from build123d import *

# Parameters (mm, degrees)
BASE_PLATE_DEPTH            = 7
ANGLED_BLOCK_DEPTH          = 50
BLOCK_NOTCH_CUT_DEPTH       = 74.464277033
BLOCK_NOTCH_CUT_DEPTH_BACK  = 74.464277033
BLOCK_RECESS_CUT_DEPTH      = 72.480306495
BLOCK_RECESS_CUT_DEPTH_BACK = 13
BLOCK_RECESS_SKETCH_R       = 4


with BuildPart() as part:
    # Base Plate Sketch → Base Plate (new body)
    with BuildSketch(Plane.XY):
        Polygon((-44, 25), (-38, 31), (38, 31), (44, 25), (44, -25), (38, -31), (-38, -31), (-44, -25), align=None)
        with BuildLine():
            Line((-30, 20.5), (-30, -20.5))
            ThreePointArc((-30, -20.5), (-33, -23.5), (-36, -20.5))
            Line((-36, -20.5), (-36, 20.5))
            ThreePointArc((-36, 20.5), (-33, 23.5), (-30, 20.5))
        make_face(mode=Mode.SUBTRACT)
        with BuildLine():
            Line((36, 20.5), (36, -20.5))
            ThreePointArc((36, -20.5), (33, -23.5), (30, -20.5))
            Line((30, -20.5), (30, 20.5))
            ThreePointArc((30, 20.5), (33, 23.5), (36, 20.5))
        make_face(mode=Mode.SUBTRACT)
    extrude(amount=BASE_PLATE_DEPTH)

    # Angled Block Sketch → Angled Block (add)
    with BuildSketch(Plane.XY):
        Polygon((-19.704957389, -4.000247215), (-12.317392569, -15.892424729), (23.166882613, 6.150837127), (15.779317794, 18.043014641), align=None)
    extrude(amount=ANGLED_BLOCK_DEPTH)

    # Block Notch Sketch → Block Notch Cut (cut, two sides: drawn at the far end of the back side and taken through both)
    with BuildSketch(Plane(origin=(0, 0, 0), x_dir=(0.8494412510349073, 0.5276832014004726, 0), z_dir=(0.5276832014004726, -0.8494412510349073, 0)).offset(-BLOCK_NOTCH_CUT_DEPTH_BACK)):
        Polygon((-18.849066913, 50), (-18.849066913, 7), (22.924599176, 42.643551505), (22.924599176, 50), align=None)
        Polygon((10.753136621, 27), (10.753136621, 7), (15.483777963, 7), (22.924599176, 7), (22.924599176, 37.385350224), align=None)
    extrude(amount=BLOCK_NOTCH_CUT_DEPTH + BLOCK_NOTCH_CUT_DEPTH_BACK, mode=Mode.SUBTRACT)

    # Block Recess Sketch → Block Recess Cut (cut, two sides: drawn at the far end of the back side and taken through both)
    with BuildSketch(Plane(origin=(-9.681672009, -6.014372005, 13.357913864), x_dir=(0.8342680576474281, -0.22636189915410374, 0.5027495386378142), z_dir=(-0.5513590554159673, -0.3425109283644645, 0.7607164096834806)).offset(-BLOCK_RECESS_CUT_DEPTH_BACK)):
        with Locations(Location((29.524664999, 24.110272289, 0), (0, 0, 193.941739612))):
            Circle(BLOCK_RECESS_SKETCH_R)
        with BuildLine():
            ThreePointArc((36.524664999, 24.110272289), (35.848943941, 21.109689701), (33.952237609, 18.688409068))
            Line((33.952237609, 18.688409068), (39.374100831, 23.115981696))
            Line((39.374100831, 23.115981696), (34.946528251, 28.53784486))
            ThreePointArc((34.946528251, 28.53784486), (36.118337828, 26.460480496), (36.524664999, 24.110272289))
        make_face()
        with BuildLine():
            Line((30.518955591, 33.959708121), (25.097092428, 29.532135541))
            ThreePointArc((25.097092428, 29.532135541), (30.227734682, 31.07487515), (34.946528251, 28.53784486))
            Line((34.946528251, 28.53784486), (30.518955591, 33.959708121))
        make_face()
    extrude(amount=BLOCK_RECESS_CUT_DEPTH + BLOCK_RECESS_CUT_DEPTH_BACK, mode=Mode.SUBTRACT)


solid = part.part
Geometry check sheet. Reference: the model listing, model coordinates, mm. A direction names the side the tool comes from. Coordinates: 2 decimals unless noted, no trailing zeros. Loops run counter-clockwise (first coordinate to the right, second up) from the corner with the lowest first, then second, coordinate; pieces in that order, holes last. Notation, with made-up numbers: (8, 40) - (49, 40) arc R19 ccw to (49, 59) - close; hole circle Ø3 at (-34.75, 22). An arc over 180 degrees is marked (long way). Use one line per item in the form item = value. Start each with the question number.
Item 1: Section check D-D, the plane y = -13. Enter the section's corners in (x, z), and give its area (3 significant figures).
Item 2: Thickness scan on probe 1 along X at (y, z) = (16, 2.5); probe 2 along Z at (x, y) = (-35.5, -26.5); probe 3 along X at (y, z) = (-7, 8). Record the ranges inside material, lowest first.
Item 3: Section check A-A, the plane y = 18.5. Enter the section's corners in (x, z), and give its area (3 significant figures).
Item 4: Section check C-C, the plane x = -9. Enter the section's corners in (y, z), and give its area (3 significant figures).
Item 5: Section check B-B, the plane x = 33. Enter the section's corners in (y, z).
Item 6: Mould release check, pull along Z, two halves, no side actions. Record for faces 1 (the face through (-1, 0, 0)), 2 (the face through (-44, 0, 3)), 3 (the face through (9.08, 5.76, 17.14)): +Z half, -Z half, draft (parallel to the pull), parting line (faces both ways), or undercut.
Item 7: Gauge pin test, flat ends, axial feed: pin 1 (1 mm diameter, centred on x = 18.5, y = 19, fed in from +Z); pin 2 (4 mm diameter, centred on y = 13.5, z = 23, fed in from +X). Record the tip position at first contact, or that the pin passes through.
Item 8: Tool access check on faces 4 (the face through (4.034, -5.735, 15.421)), 5 (the face through (-2.89, 6.446, 15.421)), 6 (the face through (-30, 0, 3)). Record the directions out of +Z, -Z, +X, -X, +Y, -Y that give a thin tool (end or side, any length) a straight path to the whole face; none if there is none.
Computed:
q1.outline = (-44, 0) - (-36, 0) - (-36, 7) - (-44, 7) - close; (-30, 0) - (30, 0) - (30, 7) - (-7.66, 7) - (-7.66, 11.68) - (-14.11, 7) - (-30, 7) - close; (36, 0) - (44, 0) - (44, 7) - (36, 7) - close
q1.area = 547 mm2
q2.probe_1 = -44 to -36, -30 to 30, 36 to 44
q2.probe_2 = 0 to 7
q2.probe_3 = -16.46 to 2
q3.outline = (-44, 0) - (-36, 0) - (-36, 7) - (-44, 7) - close; (-30, 0) - (30, 0) - (30, 7) - (-30, 7) - close; (36, 0) - (44, 0) - (44, 7) - (36, 7) - close
q3.area = 532 mm2
q4.outline = (-31, 0) - (31, 0) - (31, 7) - (2.65, 7) - (2.65, 17.75) - (-13.83, 10.33) - (-13.83, 7) - (-31, 7) - close
q4.area = 550 mm2
q5.outline = (-31, 0) - (-23.5, 0) - (-23.5, 7) - (-31, 7) - close; (23.5, 0) - (31, 0) - (31, 7) - (23.5, 7) - close
q6.face_1 = -Z half
q6.face_2 = draft
q6.face_3 = undercut
q7.pin_1 = 7
q7.pin_2 = 5.52
q8.face_4 = +Z, +X, -Y
q8.face_5 = +Z, -X, +Y
q8.face_6 = +Z, -Z
